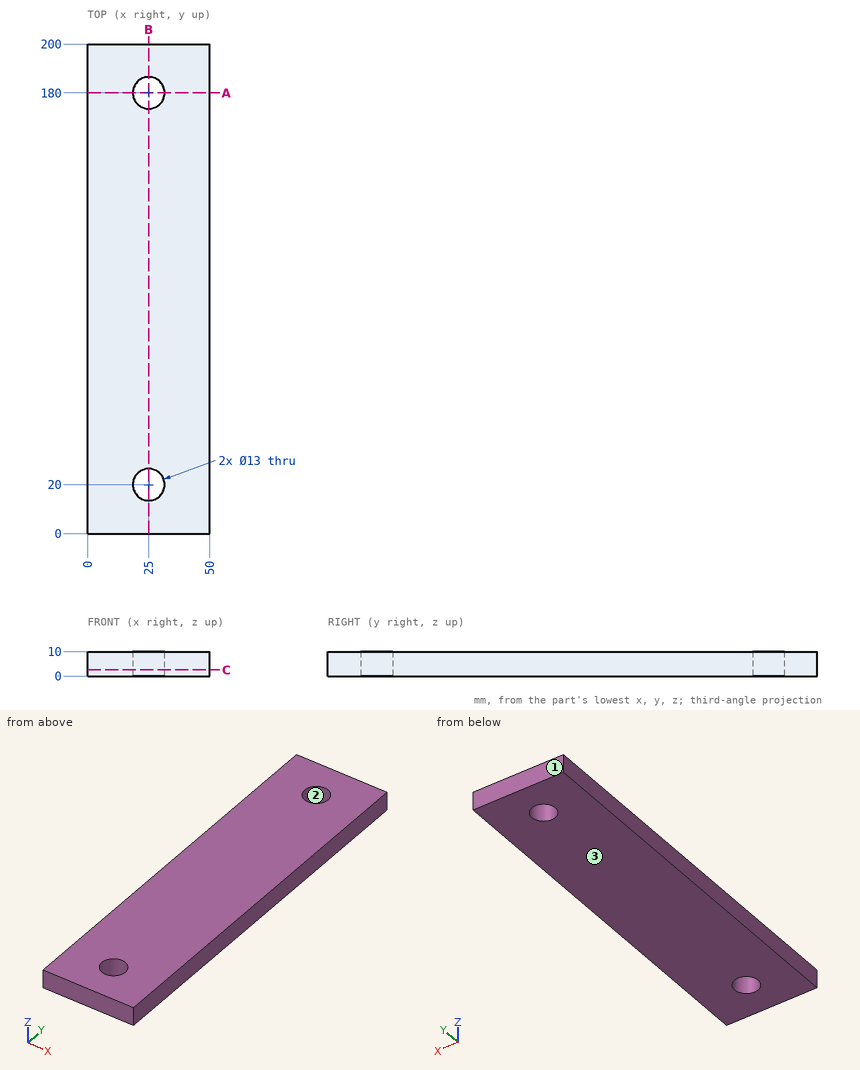
Drawing for the job (mm, zero at the part's lowest x, y, z). Round coordinates to 2 decimals unless told otherwise and drop trailing zeros. Loops run counter-clockwise (first coordinate to the right, second up) from the corner with the lowest first, then second, coordinate; pieces in that order, holes last. Notation, with made-up numbers: (64.25, 40) -> (99.25, 40) arc R27 cw to (99.25, 64) -> close; hole circle Ø2 at (-15, 67.5). An arc over 180 degrees is marked (long way). Use one line per item in the form item = value. Start each with the question number.
Item 1: Drill centre lines: line 1 along Y through (x, z) = (25, 4.25); line 2 along Y through (x, z) = (19, 8.75); line 3 along X through (y, z) = (185.5, 6.75). Where is each one in solid material? Low to high.
Item 2: Two-plate mould, pull along Y, no slides. Class the marked faces 1, 2 and 3: released by +Y, released by -Y, zero draft, split by the parting line, or undercut.
Item 3: Band-saw the part on A-A (y = 180). List the corners of the cut face in (x, z), plus the area to 3 significant figures.
Item 4: Band-saw the part on C-C (z = 2.5). List the corners of the cut face in (x, y).
Item 5: Band-saw the part on B-B (x = 25). List the corners of the cut face in (y, z).
Data:
q1.line_1 = 0 to 13.5, 26.5 to 173.5, 186.5 to 200
q1.line_2 = 0 to 17.5, 22.5 to 177.5, 182.5 to 200
q1.line_3 = 0 to 21.54, 28.46 to 50
q2.face_1 = released by +Y
q2.face_2 = undercut
q2.face_3 = zero draft
q3.outline = (0, 0) -> (18.5, 0) -> (18.5, 10) -> (0, 10) -> close; (31.5, 0) -> (50, 0) -> (50, 10) -> (31.5, 10) -> close
q3.area = 370 mm^2
q4.outline = (0, 0) -> (50, 0) -> (50, 200) -> (0, 200) -> close; hole circle Ø13 at (25, 20); hole circle Ø13 at (25, 180)
q5.outline = (0, 0) -> (13.5, 0) -> (13.5, 10) -> (0, 10) -> close; (26.5, 0) -> (173.5, 0) -> (173.5, 10) -> (26.5, 10) -> close; (186.5, 0) -> (200, 0) -> (200, 10) -> (186.5, 10) -> close
